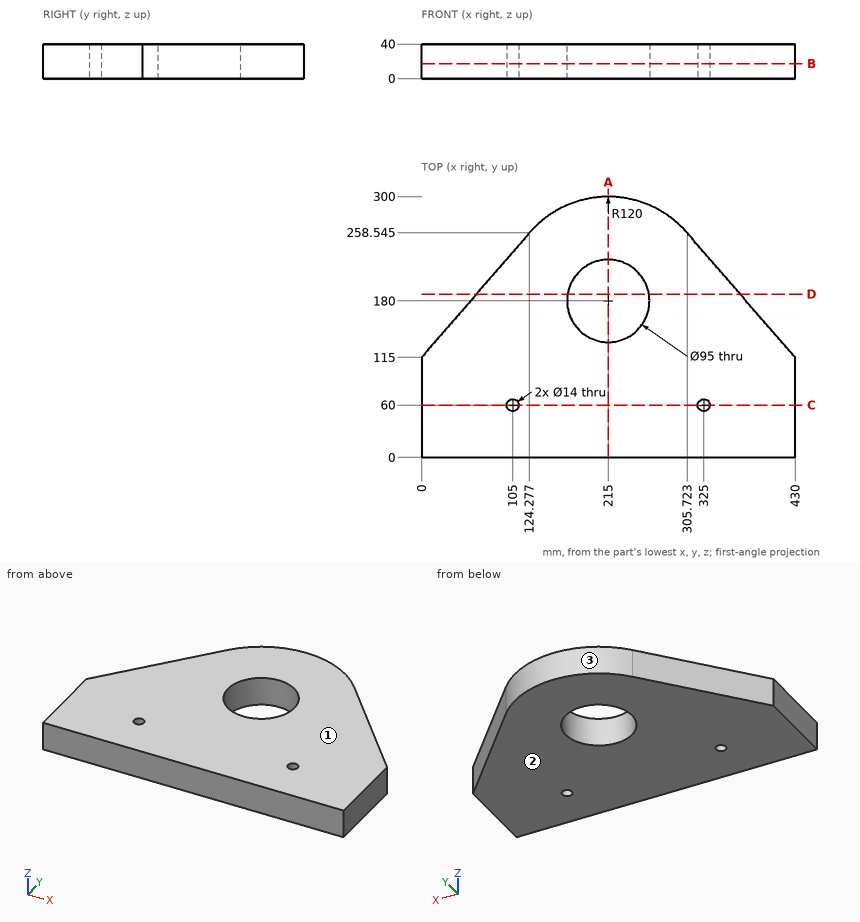
Design review of the part shown in the three views and the two pictorial views. Dimensions are in mm from the part's minimum x, y and z. Coordinates: 2 decimals unless noted, no trailing zeros. Order: outer loops, then holes, each group sorted by start corner. A loop starts at its lowest first (then second) coordinate and runs counter-clockwise, first axis right, second up.
Item 1: For pin 1 Ø6 at (x, z) = (118.5, 6.5) entering from +Y; pin 2 Ø5 at (x, z) = (106.5, 21.5) entering from +Y; pin 3 Ø1.5 at (y, z) = (142.5, 4.5) entering from -X; pin 4 Ø11 at (x, y) = (105, 60) entering from +Z, all flat-tipped, find the tip position at first contact; note any pin that passes through.
Item 2: For line 1 (Y direction, x = 105, z = 23); line 2 (X direction, y = 159.5, z = 9); line 3 (Y direction, x = 346.5, z = 16) (1 decimal), list the stretches that pass through material, from the lowest coordinate up.
Item 3: Take a section at C-C, the plane y = 60. Write out the cut boundary in (x, z), then the cut area to 3 significant figures.
Item 4: Take a section at A-A, the plane x = 215. Write out the cut boundary in (y, z).
Item 5: The part is to be moulded in two halves that separate along Z. For the marked faces 1, 2 and 3, say which applies: pulls with the +Z half, pulls with the -Z half, needs draft (parallel to the pull), parting line crosses it, or undercut.
Item 6: Take a section at D-D, the plane y = 188. Write out the cut boundary in (x, z).
Item 7: Take a section at B-B, the plane z = 17.5. Write out the cut boundary in (x, y) (1 decimal).
The answers:
1. pin 1: stops at y = 255.34
1. pin 2: stops at y = 240.9
1. pin 3: stops at x = 23.16
1. pin 4: passes through
2. line 1: y = 0 to 53, 67 to 236.28
2. line 2: x = 38.53 to 172.15, 257.85 to 391.47
2. line 3: y = 0 to 211.4
3. outline: (0, 0) - (98, 0) - (98, 40) - (0, 40) - close; (112, 0) - (318, 0) - (318, 40) - (112, 40) - close; (332, 0) - (430, 0) - (430, 40) - (332, 40) - close
3. area: 16,100 mm2
4. outline: (0, 0) - (132.5, 0) - (132.5, 40) - (0, 40) - close; (227.5, 0) - (300, 0) - (300, 40) - (227.5, 40) - close
5. face 1: pulls with the +Z half
5. face 2: pulls with the -Z half
5. face 3: needs draft
6. outline: (63.2, 0) - (168.18, 0) - (168.18, 40) - (63.2, 40) - close; (261.82, 0) - (366.8, 0) - (366.8, 40) - (261.82, 40) - close
7. outline: (0, 0) - (430, 0) - (430, 115) - (305.7, 258.5) arc R120 ccw to (124.3, 258.5) - (0, 115) - close; hole circle Ø14 at (105, 60); hole circle Ø95 at (215, 180); hole circle Ø14 at (325, 60)
